Here's how the part is built. I have some questions about the finished solid (model axes, mm). A direction names the side the tool comes from. Round coordinates to 2 decimals unless told otherwise and drop trailing zeros. Order: outer loops, then holes, each group sorted by start corner. A loop starts at its lowest first (then second) coordinate and runs counter-clockwise, first axis right, second up. Notation, with made-up numbers: (34.5, -2.5) -> (84.5, -2.5) arc R16 cw to (84.5, 4.5) -> close; hole circle Ø2 at (75.25, -11.5). An arc over 180 degrees is marked (long way). Answer in a Markdown table with one row per item.
```python
from build123d import *

# Parameters (mm, degrees)
SKETCH_1_W          = 66
SKETCH_1_H          = 10
EXTRUDE_1_DEPTH     = 190
CUT_EXTRUDE_2_DEPTH = 202.385203031
HOLE_WIZARD_M5_1_D  = 5
CUT_EXTRUDE_3_DEPTH = 202.385203031
HOLE_WIZARD_M4_1_D  = 3.3


with BuildPart() as part:
    # 草图1 → 拉伸1 (new body)
    with BuildSketch(Plane.XY):
        with Locations((33, 5)):
            Rectangle(SKETCH_1_W, SKETCH_1_H)
    extrude(amount=EXTRUDE_1_DEPTH)

    # 草图5 → 切除-拉伸2 (cut, through all)
    with BuildSketch(Plane(origin=(0, 10, 0), x_dir=(-1, 0, 0), z_dir=(0, 1, 0))):
        with BuildLine():
            Line((-43, 70), (-43, 30))
            ThreePointArc((-43, 30), (-48, 25), (-53, 30))
            Line((-53, 30), (-53, 70))
            ThreePointArc((-53, 70), (-48, 75), (-43, 70))
        make_face()
        with BuildLine():
            Line((-13, 70), (-13, 30))
            ThreePointArc((-13, 30), (-18, 25), (-23, 30))
            Line((-23, 30), (-23, 70))
            ThreePointArc((-23, 70), (-18, 75), (-13, 70))
        make_face()
        with BuildLine():
            Line((-43, 130), (-43, 90))
            ThreePointArc((-43, 90), (-48, 85), (-53, 90))
            Line((-53, 90), (-53, 130))
            ThreePointArc((-53, 130), (-48, 135), (-43, 130))
        make_face()
        with BuildLine():
            Line((-13, 130), (-13, 90))
            ThreePointArc((-13, 90), (-18, 85), (-23, 90))
            Line((-23, 90), (-23, 130))
            ThreePointArc((-23, 130), (-18, 135), (-13, 130))
        make_face()
    extrude(amount=-CUT_EXTRUDE_2_DEPTH, mode=Mode.SUBTRACT)

    # M5 螺纹孔1 (through all)
    with Locations(Plane(origin=(0, 10, 0), x_dir=(-1, 0, 0), z_dir=(0, 1, 0))):
        with Locations((-13, 10), (-53, 10)):
            Hole(HOLE_WIZARD_M5_1_D / 2)

    # 草图11 → 切除-拉伸3 (cut, through all)
    with BuildSketch(Plane(origin=(0, 10, 0), x_dir=(-1, 0, 0), z_dir=(0, 1, 0))):
        with BuildLine():
            Line((-40, 249.750844229), (-40, 170))
            ThreePointArc((-40, 170), (-33, 163), (-26, 170))
            Line((-26, 170), (-26, 249.750844229))
            Line((-26, 249.750844229), (-40, 249.750844229))
        make_face()
    extrude(amount=-CUT_EXTRUDE_3_DEPTH, mode=Mode.SUBTRACT)

    # M4 螺纹孔1 (through all)
    with Locations(Plane.XZ):
        with Locations((18, 149), (48, 149)):
            Hole(HOLE_WIZARD_M4_1_D / 2)


solid = part.part
```
1. For faces 4 (the face through (0, 5, 94)), 5 (the face through (18, 5, 135)), 6 (the face through (26, 5, 180)), which set-ups out of +Z, -Z, +X, -X, +Y, -Y let a thin tool reach every point of the face, with its end or its side?
Numbers:
| item | result |
|---|---|
| face 4 | +Z, -Z, -X, +Y, -Y |
| face 5 | +Y, -Y |
| face 6 | +Z, +Y, -Y |
2. Please list where these lines run through material, in increasing order: line 1 along X through (y, z) = (8, 129.5); line 2 along Z through (x, y) = (18, 7.5); line 3 along X through (y, z) = (5, 149).
Numbers:
| item | result |
|---|---|
| line 1 | x = 0 to 13, 23 to 43, 53 to 66 |
| line 2 | z = 0 to 25, 75 to 85, 135 to 147.35, 150.65 to 190 |
| line 3 | x = 0 to 16.35, 19.65 to 46.35, 49.65 to 66 |
3. Suppose I cut it at A-A on y = 6. State how many separate pieces and enclosed holes the cut face has, then the cut area to 3 significant figures.
Numbers:
| item | result |
|---|---|
| separate pieces | 1 |
| enclosed holes | 8 |
| area | 10,200 mm2 |
4. Suppose I cut it at C-C on z = 175. Write out the boundary of the cut face in (x, y).
Numbers:
| item | result |
|---|---|
| outline | (0, 0) -> (26, 0) -> (26, 10) -> (0, 10) -> close; (40, 0) -> (66, 0) -> (66, 10) -> (40, 10) -> close |
5. We'd pull the mould along X, two halves only. Please class faces 1 (the face through (13, 5, 190)), 2 (the face through (66, 5, 94)), 3 (the face through (23, 5, 110)): released by +X, released by -X, zero draft, split by the parting line, or undercut.
Numbers:
| item | result |
|---|---|
| face 1 | zero draft |
| face 2 | released by +X |
| face 3 | undercut |
6. Suppose I cut it at D-D on z = 97. Write out the boundary of the cut face in (x, y), then the cut area to 3 significant figures.
Numbers:
| item | result |
|---|---|
| outline | (0, 0) -> (13, 0) -> (13, 10) -> (0, 10) -> close; (23, 0) -> (43, 0) -> (43, 10) -> (23, 10) -> close; (53, 0) -> (66, 0) -> (66, 10) -> (53, 10) -> close |
| area | 460 mm2 |
7. Suppose I cut it at B-B on z = 149. Write out the boundary of the cut face in (x, y), then the cut area to 3 significant figures.
Numbers:
| item | result |
|---|---|
| outline | (0, 0) -> (16.35, 0) -> (16.35, 10) -> (0, 10) -> close; (19.65, 0) -> (46.35, 0) -> (46.35, 10) -> (19.65, 10) -> close; (49.65, 0) -> (66, 0) -> (66, 10) -> (49.65, 10) -> close |
| area | 594 mm2 |
